```python
from build123d import *

# Parameters (mm, degrees)
EXTRUDE_THIN1_DEPTH      = 18
FILLET2_R                = 1.5
FILLET3_R                = 3
BOSS_EXTRUDE1_DEPTH      = 30
BOSS_EXTRUDE1_DEPTH_BACK = 15
SKETCH5_W                = 3
SKETCH5_H                = 3
CUT_EXTRUDE2_DEPTH       = 30
CUT_EXTRUDE3_DEPTH       = 73.341205409
CUT_EXTRUDE4_DEPTH       = 10


with BuildPart() as part:
    # Sketch1 → Extrude-Thin1 (new body)
    with BuildSketch(Plane.XY):
        Polygon((25, 0), (0, 0), (0, 40), (-1.5, 40), (-1.5, -1.5), (25, -1.5), align=None)
    extrude(amount=EXTRUDE_THIN1_DEPTH)

    # Fillet2
    fillet2_edges = [part.edges().sort_by_distance(p)[0] for p in [
        (0, 0, 9),
    ]]
    fillet(fillet2_edges, radius=FILLET2_R)

    # Fillet3
    fillet3_edges = [part.edges().sort_by_distance(p)[0] for p in [
        (-1.5, -1.5, 9),
    ]]
    fillet(fillet3_edges, radius=FILLET3_R)

    # Sketch4 → Boss-Extrude1 (add, two sides: drawn at the far end of the back side and taken through both)
    with BuildSketch(Plane(origin=(25, 0, 0), x_dir=(0, 0, -1), z_dir=(1, 0, 0)).offset(-BOSS_EXTRUDE1_DEPTH_BACK)):
        with BuildLine():
            Line((-21, -3), (-21, -21))
            Line((-21, -21), (-19.5, -21))
            Line((-19.5, -21), (-19.5, -3))
            ThreePointArc((-19.5, -3), (-19.060660172, -1.939339828), (-18, -1.5))
            Line((-18, -1.5), (-18, 0))
            ThreePointArc((-18, 0), (-20.121320344, -0.878679656), (-21, -3))
        make_face()
    extrude(amount=BOSS_EXTRUDE1_DEPTH + BOSS_EXTRUDE1_DEPTH_BACK)

    # Sketch5 → Cut-Extrude2 (cut)
    with BuildSketch(Plane(origin=(55, 0, 0), x_dir=(0, 0, -1), z_dir=(1, 0, 0))):
        with Locations((-19.5, -1.5)):
            Rectangle(SKETCH5_W, SKETCH5_H)
    extrude(amount=-CUT_EXTRUDE2_DEPTH, mode=Mode.SUBTRACT)

    # Sketch6 → Cut-Extrude3 (cut, through all)
    with BuildSketch(Plane.ZY.offset(1.5)):
        with BuildLine():
            Line((6.25, 34), (6.25, 19))
            ThreePointArc((6.25, 19), (4.5, 17.25), (2.75, 19))
            Line((2.75, 19), (2.75, 34))
            ThreePointArc((2.75, 34), (4.5, 35.75), (6.25, 34))
        make_face()
        with BuildLine():
            Line((11.75, 34), (11.75, 19))
            ThreePointArc((11.75, 19), (13.5, 17.25), (15.25, 19))
            Line((15.25, 19), (15.25, 34))
            ThreePointArc((15.25, 34), (13.5, 35.75), (11.75, 34))
        make_face()
    extrude(amount=-CUT_EXTRUDE3_DEPTH, mode=Mode.SUBTRACT)

    # Sketch7 → Cut-Extrude4 (cut)
    with BuildSketch(Plane.XY.offset(21)):
        with BuildLine():
            Line((30, -5.75), (40, -5.75))
            ThreePointArc((40, -5.75), (41.75, -7.5), (40, -9.25))
            Line((40, -9.25), (30, -9.25))
            ThreePointArc((30, -9.25), (28.25, -7.5), (30, -5.75))
        make_face()
        with BuildLine():
            Line((30, -18.25), (40, -18.25))
            ThreePointArc((40, -18.25), (41.75, -16.5), (40, -14.75))
            Line((40, -14.75), (30, -14.75))
            ThreePointArc((30, -14.75), (28.25, -16.5), (30, -18.25))
        make_face()
    extrude(amount=-CUT_EXTRUDE4_DEPTH, mode=Mode.SUBTRACT)


solid = part.part
```
Design review of the part built by this model. Coordinates are the model's own, in mm. A direction names the side the tool comes from. Give positions to 0.01 mm unless a question says otherwise; leave off trailing zeros. Write each loop counter-clockwise with the first axis right and the second up, starting at its lowest first coordinate (ties: lowest second). Pieces come first, ordered by that corner, then holes.
(1) Add section D-D (z = 9.25). Give the boundary of the cut face in (x, y).
Checked values:
outline: (-1.5, 1.5) arc R3 ccw to (1.5, -1.5) - (25, -1.5) - (25, 0) - (1.5, 0) arc R1.5 cw to (0, 1.5) - (0, 40) - (-1.5, 40) - close
(2) Add section B-B (y = -16.5). Give the boundary of the cut face in (x, z), and give its area (4 significant figures).
Checked values:
outline: (10, 19.5) - (28.25, 19.5) - (28.25, 21) - (10, 21) - close; (41.75, 19.5) - (55, 19.5) - (55, 21) - (41.75, 21) - close
area: 47.25 mm2
(3) Clearance check with flat-ended pins moving along their axes: pin 1 Ø1.6 at (x, y) = (-0.5, 29) entering from +Z; pin 2 Ø3.5 at (x, y) = (2.5, 19.5) entering from +Z; pin 3 Ø10 at (y, z) = (13.5, 15.5) entering from +X; pin 4 Ø1.5 at (y, z) = (-1.5, 6.5) entering from -X. State where each tip first meets the part, or that it passes through.
Checked values:
pin 1: stops at z = 18
pin 2: passes through
pin 3: stops at x = 0
pin 4: stops at x = -0.48
(4) Wall thickness on line 1 along Y through (x, z) = (2, 6.25); line 2 along Y through (x, z) = (16, 19.25): over which ranges is each line inside the solid? List them lowest first.
Checked values:
line 1: y = -1.5 to 0
line 2: y = -2.17 to -0.27
(5) Add section A-A (z = 13.5). Give the boundary of the cut face in (x, y).
Checked values:
outline: (-1.5, 1.5) arc R3 ccw to (1.5, -1.5) - (25, -1.5) - (25, 0) - (1.5, 0) arc R1.5 cw to (0, 1.5) - (0, 17.25) - (-1.5, 17.25) - close; (-1.5, 35.75) - (0, 35.75) - (0, 40) - (-1.5, 40) - close
(6) Add section C-C (x = 37). Give the boundary of the cut face in (y, z), and give its area (3 significant figures).
Checked values:
outline: (-21, 19.5) - (-18.25, 19.5) - (-18.25, 21) - (-21, 21) - close; (-14.75, 19.5) - (-9.25, 19.5) - (-9.25, 21) - (-14.75, 21) - close; (-5.75, 19.5) - (-3, 19.5) - (-3, 21) - (-5.75, 21) - close
area: 16.5 mm2
(7) Mouldability with a two-part tool opening along X and no side actions: class faces 1 (the face through (17.4, -0.86, 20.1)), 2 (the face through (35, -18.25, 20)), 3 (the face through (-0.6, -0.64, 9.13)) as +X half, -X half, draft (parallel to the pull), parting line (faces both ways), or undercut.
Checked values:
face 1: draft
face 2: undercut
face 3: -X half
(8) Tool access review of faces 4 (the face through (10, -10, 20)), 5 (the face through (13, -1.5, 9)), 6 (the face through (-0.76, 35.75, 4.46)), 7 (the face through (35, -5.75, 20)): name each direction out of +Z, -Z, +X, -X, +Y, -Y from which nothing blocks a thin tool from reaching the whole face with its end or side.
Checked values:
face 4: +Z, -X, +Y, -Y
face 5: -Z, +X, -X, -Y
face 6: +X, -X
face 7: +Z, -Z
